Read the model definition and answer for the solid it produces. Units are mm, in the model's axes. Give positions to 0.01 mm unless a question says otherwise; leave off trailing zeros. Order: outer loops, then holes, each group sorted by start corner. A loop starts at its lowest first (then second) coordinate and runs counter-clockwise, first axis right, second up.
Item 1: Given pin 1 Ø3 at (x, z) = (40, -23) entering from -Y, flat-ended and moving along its own axis, determine where the tip first touches the part or whether it passes through.
Item 2: A cutting plane is placed at B-B (x = 40). Write down the section's boundary in (y, z).
Item 3: The mould has two halves that part along X. Classify faces 1 (the face through (40.9, 16.7, -24.5)), 2 (the face through (-42.5, 16, 0)), 3 (the face through (-1, 33, 0)): +X half, -X half, draft (parallel to the pull), parting line (faces both ways), or undercut.
Item 4: Find the intervals of material crossed by line 1 along X through (y, z) = (17, -23); line 2 along Z through (x, y) = (40, 9.5); line 3 along X through (y, z) = (16, 24), in increasing order.
Item 5: A cutting plane is placed at A-A (z = -23). Write down the section's boundary in (x, y), plus the area to 3 significant figures.
from build123d import *

# Parameters (mm, degrees)
SKETCH_1_W              = 85
SKETCH_1_H              = 58
EXTRUDE_1_DEPTH         = 33
HOLE_WIZARD_3_5_3_5_1_D = 3.5


with BuildPart() as part:
    # 草图1 → 凸台-拉伸1 (new body)
    with BuildSketch(Plane(origin=(0, 0, 0), x_dir=(1, 0, 0), z_dir=(0, 1, 0))):
        Rectangle(SKETCH_1_W, SKETCH_1_H)
    extrude(amount=EXTRUDE_1_DEPTH)

    # Ø3.5 (3.5) 直径孔1 (through all)
    with Locations(Plane(origin=(0, 0, 0), x_dir=(-1, 0, 0), z_dir=(0, -1, 0))):
        with Locations((39, -24), (-40, 23)):
            Hole(HOLE_WIZARD_3_5_3_5_1_D / 2)


solid = part.part
Response values:
1. pin 1: passes through
2. outline: (0, -29) - (33, -29) - (33, -24.75) - (0, -24.75) - close; (0, -21.25) - (33, -21.25) - (33, 29) - (0, 29) - close
3. face 1: undercut
3. face 2: -X half
3. face 3: draft
4. line 1: x = -42.5 to 38.25, 41.75 to 42.5
4. line 2: z = -29 to -24.75, -21.25 to 29
4. line 3: x = -42.5 to -40.75, -37.25 to 42.5
5. outline: (-42.5, 0) - (38.25, 0) - (38.25, 33) - (-42.5, 33) - close; (41.75, 0) - (42.5, 0) - (42.5, 33) - (41.75, 33) - close
5. area: 2,690 mm2
